Study the drawing (mm; zero at the part's minimum x, y, z) and answer. Give positions to 0.01 mm unless a question says otherwise; leave off trailing zeros. Order: outer loops, then holes, each group sorted by start corner. A loop starts at its lowest first (then second) coordinate and runs counter-clockwise, first axis right, second up. Notation, with made-up numbers: (19.5, 24) - (78.5, 24) arc R11 ccw to (78.5, 35) - close; hole circle Ø8 at (-4.5, 75.25). An arc over 180 degrees is marked (long way). Write each question's results on one line, items separated by ' | '. Start each with the question number.
Q1. For a pull along X with two mould halves and no side action, classify the marked faces 1 and 2 as +X half, -X half, draft (parallel to the pull), parting line (faces both ways), or undercut.
Q2. Find section B-B on x = 5. Give the vertices of the cut face in (y, z).
Q3. Find the intervals of material crossed by line 1 along Y through (x, z) = (95, 18); line 2 along X through (y, z) = (6.5, 25); line 3 along Y through (x, z) = (39.5, 19), in increasing order. Write a range as from..to.
Q4. Find section A-A on z = 26.5. Give the vertices of the cut face in (x, y).
Q5. Flat-ended cylindrical pins translate along their axes: P1, Ø1.2, axis at y = 5, z = 10.5, coming from the +X side; P2, Ø2, axis at y = 5, z = 10, coming from the -X side; P3, Ø2, axis at x = 21.5, z = 19.5, coming from the +Y side; P4, Ø5, axis at x = 28, y = 5.5, coming from the +Z side. Find the tip coordinate at first contact, or state that the pin passes through.
Q6. Find section C-C on x = 52. Give the vertices of the cut face in (y, z), and give its area (3 significant figures).
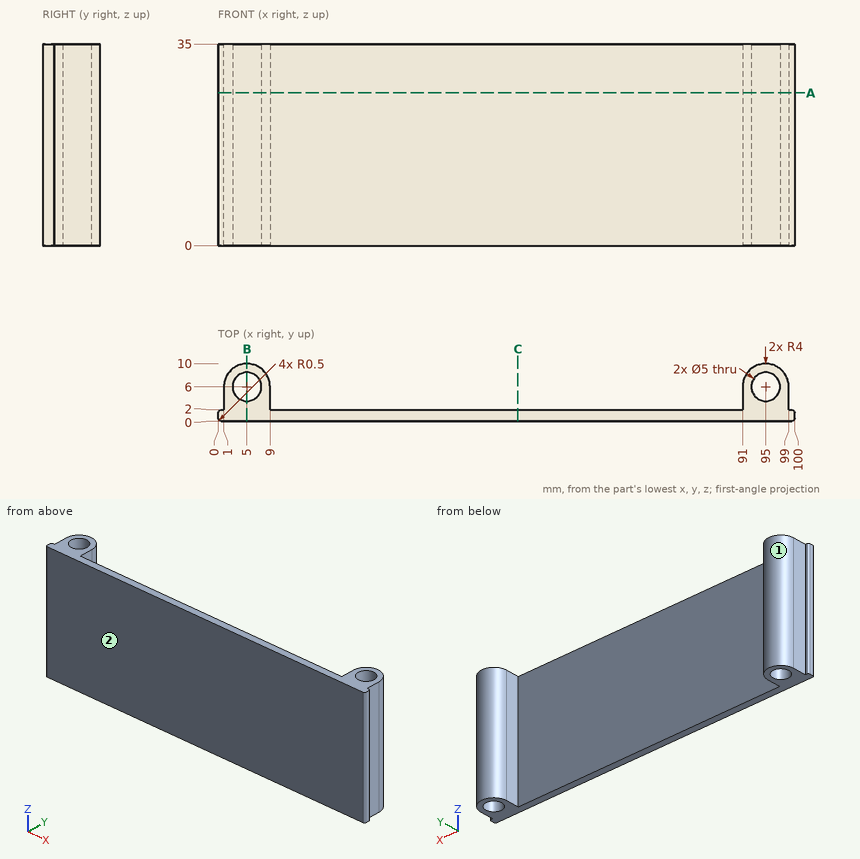
Working result:
1) face 1: undercut | face 2: draft
2) outline: (0, 0) - (3.5, 0) - (3.5, 35) - (0, 35) - close; (8.5, 0) - (10, 0) - (10, 35) - (8.5, 35) - close
3) line 1: 0..3.5, 8.5..10 | line 2: 1.03..2.55, 7.45..8.97, 91.03..92.55, 97.45..98.97 | line 3: 0..2
4) outline: (0, 0.5) arc R0.5 ccw to (0.5, 0) - (99.5, 0) arc R0.5 ccw to (100, 0.5) - (100, 1.5) arc R0.5 ccw to (99.5, 2) - (99, 2) - (99, 6) arc R4 ccw to (91, 6) - (91, 2) - (9, 2) - (9, 6) arc R4 ccw to (1, 6) - (1, 2) - (0.5, 2) arc R0.5 ccw to (0, 1.5) - close; hole circle Ø5 at (5, 6); hole circle Ø5 at (95, 6)
5) P1: x = 99 | P2: x = 1 | P3: y = 2 | P4: through
6) outline: (0, 0) - (2, 0) - (2, 35) - (0, 35) - close | area: 70.0 mm²
